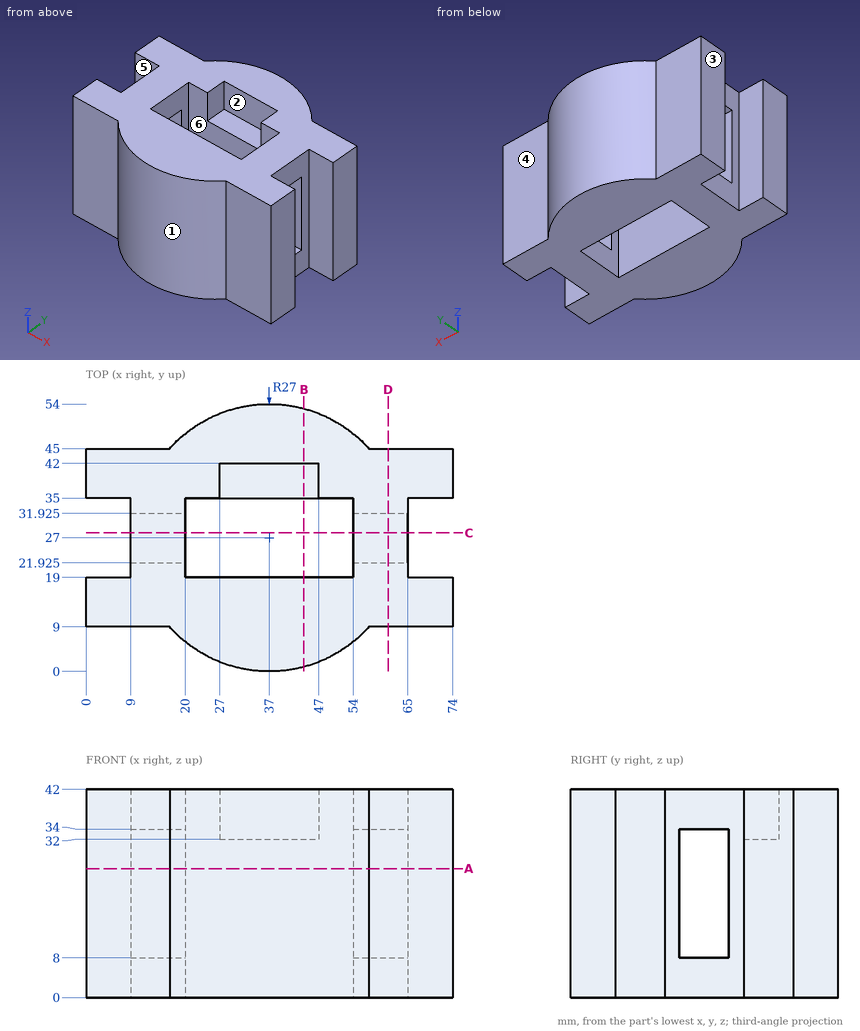
Geometry check sheet. Reference: drawing and pictorial views, mm from the part's lowest x, y, z. A direction names the side the tool comes from. Round coordinates to 2 decimals unless told otherwise and drop trailing zeros. Order: outer loops, then holes, each group sorted by start corner. A loop starts at its lowest first (then second) coordinate and runs counter-clockwise, first axis right, second up.
Q1. Cross-section at B-B, the plane x = 44. Enter the section's corners in (y, z).
Filled sheet:
outline: (0.92, 0) - (19, 0) - (19, 42) - (0.92, 42) - close; (35, 0) - (53.08, 0) - (53.08, 42) - (42, 42) - (42, 32) - (35, 32) - close
Q2. Depth check by flat-ended pin: P1, Ø2, axis at x = 52.5, z = 12, coming from the -Y side; P2, Ø6, axis at x = 32.5, z = 7.5, coming from the -Y side; P3, Ø18.5, axis at x = 64.5, z = 31.5, coming from the -Y side. Enter the tip coordinate at first touch or a pass-through.
Filled sheet:
P1: stops at y = 4.22
P2: stops at y = 0.04
P3: stops at y = 7.1
Q3. Set-up check for the marked faces 4, 5 and 6: record each of +Z, -Z, +X, -X, +Y, -Y from which the full face is reachable in a straight line by a thin tool's end or side.
Filled sheet:
face 4: +Z, -Z, +X, +Y
face 5: +Z, -Z, -X
face 6: +Z, -Z
Q4. Draft check along Y on the marked faces 1, 2 and 3. Enter one of: pulls with the +Y half, pulls with the -Y half, needs draft (parallel to the pull), parting line crosses it, or undercut.
Filled sheet:
face 1: pulls with the -Y half
face 2: undercut
face 3: needs draft
Q5. Cross-section at A-A, the plane z = 26. Enter the section's corners in (x, y) (1 decimal).
Filled sheet:
outline: (0, 9) - (16.9, 9) arc R27 ccw to (57.1, 9) - (74, 9) - (74, 19) - (65, 19) - (65, 21.9) - (54, 21.9) - (54, 19) - (20, 19) - (20, 21.9) - (9, 21.9) - (9, 19) - (0, 19) - close; (0, 35) - (9, 35) - (9, 31.9) - (20, 31.9) - (20, 35) - (54, 35) - (54, 31.9) - (65, 31.9) - (65, 35) - (74, 35) - (74, 45) - (57.1, 45) arc R27 ccw to (16.9, 45) - (0, 45) - close
Q6. Scan lines: L1, parallel to Z at x = 56.5, y = 26; L2, parallel to Y at x = 38, z = 17; L3, parallel to Y at x = 69, z = 26.5. Record each from-to range of solid material in increasing order.
Filled sheet:
L1: z = 0 to 8, 34 to 42
L2: y = 0.02 to 19, 35 to 53.98
L3: y = 9 to 19, 35 to 45
Q7. Cross-section at D-D, the plane x = 61. Enter the section's corners in (y, z) (1 decimal).
Filled sheet:
outline: (9, 0) - (45, 0) - (45, 42) - (9, 42) - close; hole (21.9, 8) - (31.9, 8) - (31.9, 34) - (21.9, 34) - close
Q8. Cross-section at C-C, the plane y = 28. Enter the section's corners in (x, z), plus the area to 3 significant figures.
Filled sheet:
outline: (9, 0) - (20, 0) - (20, 8) - (9, 8) - close; (9, 34) - (20, 34) - (20, 42) - (9, 42) - close; (54, 0) - (65, 0) - (65, 8) - (54, 8) - close; (54, 34) - (65, 34) - (65, 42) - (54, 42) - close
area: 352 mm2
